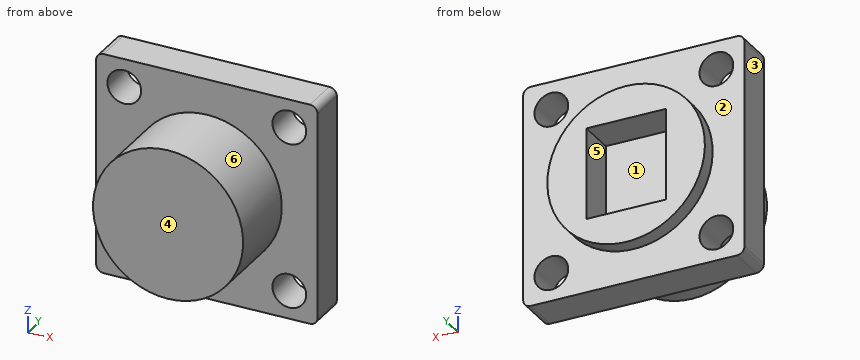
```python
from build123d import *

# Parameters (mm, degrees)
SKETCH_1_R          = 10
EXTRUDE_1_DEPTH     = 10
SKETCH_2_W          = 29.5
SKETCH_2_H          = 29.5
EXTRUDE_2_DEPTH     = 5
SKETCH_3_R          = 10.5
EXTRUDE_3_DEPTH     = 17
SKETCH_4_R          = 2.25
CUT_EXTRUDE_1_DEPTH = 17
FILLET_1_R          = 1
CUT_EXTRUDE_START   = -15
SKETCH_5_R          = 10.5
CUT_EXTRUDE_2_DEPTH = 15
SKETCH_6_W          = 10.574518314
SKETCH_6_H          = 12.201367284
CUT_EXTRUDE_3_DEPTH = 5


with BuildPart() as part:
    # 草图1 → 凸台-拉伸1 (new body)
    with BuildSketch(Plane(origin=(0, 0, 0), x_dir=(1, 0, 0), z_dir=(0, 1, 0))):
        with Locations(Location((0, 0, 0), (0, 0, 270))):
            Circle(SKETCH_1_R)
    extrude(amount=EXTRUDE_1_DEPTH)

    # 草图2 → 凸台-拉伸2 (add)
    with BuildSketch(Plane(origin=(0, 10, 0), x_dir=(1, 0, 0), z_dir=(0, 1, 0))):
        Rectangle(SKETCH_2_W, SKETCH_2_H)
    extrude(amount=EXTRUDE_2_DEPTH)

    # 草图3 → 凸台-拉伸3 (add)
    with BuildSketch(Plane(origin=(0, 15, 0), x_dir=(1, 0, 0), z_dir=(0, 1, 0))):
        with Locations(Location((0, 0, 0), (0, 0, 270))):
            Circle(SKETCH_3_R)
    extrude(amount=EXTRUDE_3_DEPTH)

    # 草图4 → 切除-拉伸1 (cut)
    with BuildSketch(Plane(origin=(0, 15, 0), x_dir=(1, 0, 0), z_dir=(0, 1, 0))):
        with Locations(Location((11, 11, 0), (0, 0, 270))):
            Circle(SKETCH_4_R)
        with Locations(Location((-11, 11, 0), (0, 0, 270))):
            Circle(SKETCH_4_R)
        with Locations(Location((-11, -11, 0), (0, 0, 270))):
            Circle(SKETCH_4_R)
        with Locations(Location((11, -11, 0), (0, 0, 270))):
            Circle(SKETCH_4_R)
    extrude(amount=-CUT_EXTRUDE_1_DEPTH, mode=Mode.SUBTRACT)

    # 圆角1
    fillet_1_edges = [part.edges().sort_by_distance(p)[0] for p in [
        (14.75, 12.5, 14.75),
        (14.75, 12.5, -14.75),
        (-14.75, 12.5, -14.75),
        (-14.75, 12.5, 14.75),
    ]]
    fillet(fillet_1_edges, radius=FILLET_1_R)

    # 草图5 → 切除-拉伸2 (cut)
    with BuildSketch(Plane(origin=(0, 32, 0), x_dir=(1, 0, 0), z_dir=(0, 1, 0)).offset(CUT_EXTRUDE_START)):
        with Locations(Location((0, 0, 0), (0, 0, 270))):
            Circle(SKETCH_5_R)
    extrude(amount=CUT_EXTRUDE_2_DEPTH, mode=Mode.SUBTRACT)

    # 草图6 → 切除-拉伸3 (cut)
    with BuildSketch(Plane(origin=(0, 17, 0), x_dir=(1, 0, 0), z_dir=(0, 1, 0))):
        Rectangle(SKETCH_6_W, SKETCH_6_H)
    extrude(amount=-CUT_EXTRUDE_3_DEPTH, mode=Mode.SUBTRACT)


solid = part.part
```
Geometry: final body of the model. Coordinates: model frame, mm. Face numbers are marked on the shaded views. A direction names the side the tool comes from. Round coordinates to 2 decimals unless told otherwise and drop trailing zeros. Order: outer loops, then holes, each group sorted by start corner. A loop starts at its lowest first (then second) coordinate and runs counter-clockwise, first axis right, second up. Notation, with made-up numbers: (48, 3) - (75, 3) arc R24 cw to (75, 33) - close; hole circle Ø6 at (-28.75, 57.5). An arc over 180 degrees is marked (long way). Write item = value, one per line. Start each with the question number.
Q1. Cut plane A-A on x = 0. Return the cut outline in (y, z).
Q2. Cut plane C-C on x = 11. Return the cut outline in (y, z), and give its area (4 significant figures).
Q3. Pull-direction query (X, two-part tool) for the marked faces 1, 2 and 3; classes: +X half, -X half, draft (parallel to the pull), parting line (faces both ways), or undercut.
Q4. Access query for the marked faces 4, 5 and 6. Directions: +Z, -Z, +X, -X, +Y, -Y. A direction counts if a zero-diameter tool reaches every point of the face in a straight line with its end or side. Return the directions, or none.
Q5. Pin query (flat end, axial travel): pin 1 (2 mm diameter, centred on x = 2, z = 0.5, fed in from +Y); pin 2 (1.5 mm diameter, centred on x = -8.5, z = 2.5, fed in from -Y); pin 3 (7 mm diameter, centred on x = -11, z = 11, fed in from +Y); pin 4 (10 mm diameter, centred on x = 3, y = 2.5, fed in from -Z). Return the tip coordinate at first contact, or that it passes through.
Q6. Ray query, line 1 (X direction, y = 12.35, z = -11); line 2 (Z direction, x = -4.5, y = 12.25); line 3 (Y direction, x = 6.75, z = 11.25). Return the intervals inside material, ascending. Write a range as from..to.
Q7. Cut plane B-B on z = -11. Return the cut outline in (x, y), and give its area (4 significant figures).
Q8. Cut plane D-D on y = 16.25. Return the cut outline in (x, z), and give its area (3 significant figures).
Outcome:
q1.outline = (0, -10) - (10, -10) - (10, -14.75) - (15, -14.75) - (15, -10.5) - (17, -10.5) - (17, -6.1) - (12, -6.1) - (12, 6.1) - (17, 6.1) - (17, 10.5) - (15, 10.5) - (15, 14.75) - (10, 14.75) - (10, 10) - (0, 10) - close
q2.outline = (10, -14.75) - (15, -14.75) - (15, -13.25) - (10, -13.25) - close; (10, -8.75) - (15, -8.75) - (15, 8.75) - (10, 8.75) - close; (10, 13.25) - (15, 13.25) - (15, 14.75) - (10, 14.75) - close
q2.area = 102.5 mm^2
q3.face_1 = undercut
q3.face_2 = draft
q3.face_3 = -X half
q4.face_4 = +Z, -Z, +X, -X, -Y
q4.face_5 = +Y
q4.face_6 = -Y
q5.pin_1 = 12
q5.pin_2 = 0
q5.pin_3 = 15
q5.pin_4 = -10
q6.line_1 = -14.75..-13.25, -8.75..8.75, 13.25..14.75
q6.line_2 = -14.75..-6.1, 6.1..14.75
q6.line_3 = 10..15
q7.outline = (-14.75, 10) - (-13.25, 10) - (-13.25, 15) - (-14.75, 15) - close; (-8.75, 10) - (8.75, 10) - (8.75, 15) - (-8.75, 15) - close; (13.25, 10) - (14.75, 10) - (14.75, 15) - (13.25, 15) - close
q7.area = 102.5 mm^2
q8.outline = circle Ø21 at (0, 0); hole (-5.29, -6.1) - (5.29, -6.1) - (5.29, 6.1) - (-5.29, 6.1) - close
q8.area = 217 mm^2
